from build123d import *

# Parameters (mm, degrees)
EXTRUDE_1_DEPTH              = 13.6
CHAMFER_1_SIZE               = 0.5
HOLE_WIZARD_M4_1_D           = 4.5
HOLE_WIZARD_M4_1_CBORE_D     = 8
HOLE_WIZARD_M4_1_CBORE_DEPTH = 4.4
SKETCH_6_W                   = 2
SKETCH_6_H                   = 15
EXTRUDE_2_DEPTH              = 13.6
HOLE_WIZARD_M3_1_D           = 2.5
MM_1_D                       = 4
MM_1_DEPTH                   = 10
MM_1_TIP                     = 1.201721238
CHAMFER_2_SIZE               = 0.5
MM_2_D                       = 3
MM_2_DEPTH                   = 1
MM_2_TIP                     = 0.901290929


with BuildPart() as part:
    # 草图3 → 凸台-拉伸1 (new body)
    with BuildSketch(Plane.XY):
        Polygon((10, 37.5), (9.5, 38), (-9.5, 38), (-10, 37.5), (-10, 23.5), (-9.5, 23), (-2, 23), (-2, 8), (-9.5, 8), (-10, 7.5), (-10, -7.5), (-9.5, -8), (-2, -8), (-2, -23), (-9.5, -23), (-10, -23.5), (-10, -37.5), (-9.5, -38), (9.5, -38), (10, -37.5), align=None)
    extrude(amount=-EXTRUDE_1_DEPTH)

    # 倒角1
    chamfer_1_edges = [part.edges().sort_by_distance(p)[0] for p in [
        (-10, 30.5, -13.6),
        (-9.75, 37.75, -13.6),
        (0, 38, -13.6),
        (9.75, 37.75, -13.6),
        (10, 0, -13.6),
        (9.75, -37.75, -13.6),
        (-10, -30.5, -13.6),
        (-9.75, -37.75, -13.6),
        (0, -38, -13.6),
        (-10, 30.5, 0),
        (-9.75, 37.75, 0),
        (0, 38, 0),
        (9.75, 37.75, 0),
        (10, 0, 0),
        (9.75, -37.75, 0),
        (-10, -30.5, 0),
        (-9.75, -37.75, 0),
        (0, -38, 0),
    ]]
    chamfer(chamfer_1_edges, length=CHAMFER_1_SIZE)

    # M4 六角凹头螺钉的柱形沉头孔1 (through all)
    with Locations(Plane.ZY.offset(10)):
        with Locations((-6.8, -30), (-6.8, 30)):
            CounterBoreHole(HOLE_WIZARD_M4_1_D / 2, HOLE_WIZARD_M4_1_CBORE_D / 2, HOLE_WIZARD_M4_1_CBORE_DEPTH)

    # 草图6 → 凸台-拉伸2 (add)
    with BuildSketch(Plane.XY):
        with Locations((-3, -15.5)):
            Rectangle(SKETCH_6_W, SKETCH_6_H)
        with Locations((-3, 15.5)):
            Rectangle(SKETCH_6_W, SKETCH_6_H)
    extrude(amount=-EXTRUDE_2_DEPTH)

    # M3 螺纹孔1 (through all)
    with Locations(Plane.ZY.offset(4)):
        with Locations((-6.8, -15.5), (-6.8, 15.5)):
            Hole(HOLE_WIZARD_M3_1_D / 2)

    # 大小mm 暗销孔1
    with Locations(Plane(origin=(10, 0, 0), x_dir=(0, 0, -1), z_dir=(1, 0, 0))):
        with Locations((6.8, -23), (6.8, 23)):
            Hole(MM_1_D / 2, depth=MM_1_DEPTH)
            with Locations((0, 0, -(MM_1_DEPTH + MM_1_TIP / 2))):  # 118° drill point
                Cone(0, MM_1_D / 2, MM_1_TIP, mode=Mode.SUBTRACT)

    # 倒角2
    chamfer_2_edges = [part.edges().sort_by_distance(p)[0] for p in [
        (-10, 30, -10.8),
        (10, 30, -4.55),
        (-10, -30, -10.8),
        (10, -30, -4.55),
        (10, 15.5, -5.55),
        (10, -15.5, -5.55),
        (10, 23, -8.8),
        (10, -23, -8.8),
    ]]
    chamfer(chamfer_2_edges, length=CHAMFER_2_SIZE)

    # 大小mm 暗销孔2
    with Locations(Plane.ZY.offset(10)):
        with Locations((-6.8, 0)):
            Hole(MM_2_D / 2, depth=MM_2_DEPTH)
            with Locations((0, 0, -(MM_2_DEPTH + MM_2_TIP / 2))):  # 118° drill point
                Cone(0, MM_2_D / 2, MM_2_TIP, mode=Mode.SUBTRACT)


solid = part.part
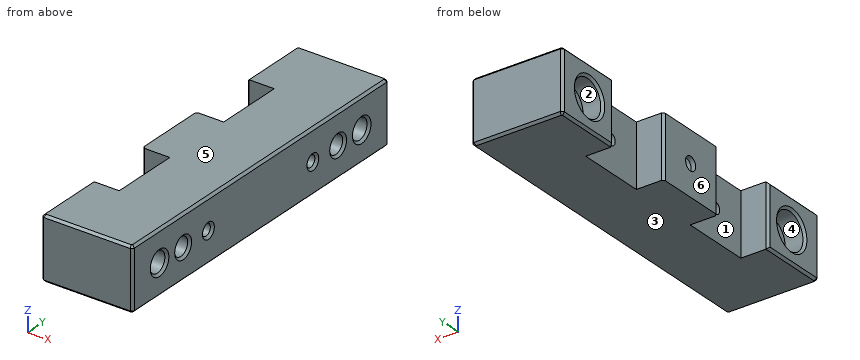
Part model, mm, in its own coordinate system. Face numbers are marked on the shaded views. A direction names the side the tool comes from. Coordinates: 2 decimals unless noted, no trailing zeros. Write each loop counter-clockwise with the first axis right and the second up, starting at its lowest first coordinate (ties: lowest second). Pieces come first, ordered by that corner, then holes. Notation, with made-up numbers: M -17.75,82 L 36.25,82 A23 ccw 36.25,100 Z; hole C 47,66 d1. An arc over 180 degrees is marked long. Return JSON: item names as keys, results as strings.
1. Probe L1, parallel to Y at x = -1.5, z = -6.8; L2, parallel to Y at x = -6.75, z = -6.8; L3, parallel to Z at x = 3.5, y = -23. List the from-to ranges inside material, lowest first.
Determined:
{"L1": "-38 to -32.25, -27.75 to -16.75, -14.25 to 14.25, 16.75 to 27.75, 32.25 to 38", "L2": "-38 to -34, -26 to -23, -8 to 8, 23 to 26, 34 to 38", "L3": "-13.6 to -8.8, -4.8 to 0"}
2. Flat gauge pins, fed straight in: pin 1 Ø3 at (y, z) = (-15.5, -6.8) entering from +X; pin 2 Ø2.5 at (y, z) = (-28, -6) entering from -X; pin 3 Ø4 at (y, z) = (-18.5, -7.5) entering from -X. Where does each tip first touch, or does it go through?
Determined:
{"pin 1": "x = 9.75", "pin 2": "x = -5.6", "pin 3": "x = -4"}
3. Pull direction Z, two halves, no side cores. Call the marked faces 4, 5 and 6: pulls with the +Z half, pulls with the -Z half, needs draft (parallel to the pull), parting line crosses it, or undercut.
Determined:
{"face 4": "undercut", "face 5": "pulls with the +Z half", "face 6": "needs draft"}
4. Saw through at B-B, the plane x = 4. Write the cut outline in (y, z), then the cut area to 3 significant figures.
Determined:
{"outline": "M -38,-13.1 L -37.5,-13.6 L 37.5,-13.6 L 38,-13.1 L 38,-0.5 L 37.5,0 L -37.5,0 L -38,-0.5 Z; hole C -30,-6.8 d4.5; hole C -23,-6.8 d4; hole C -15.5,-6.8 d2.5; hole C 15.5,-6.8 d2.5; hole C 23,-6.8 d4; hole C 30,-6.8 d4.5", "area": "966 mm²"}
5. Saw through at A-A, the plane y = -30. Write the cut outline in (x, z).
Determined:
{"outline": "M -10,-13.1 L -9.5,-13.6 L 9.5,-13.6 L 10,-13.1 L 10,-9.55 L 9.5,-9.05 L -5.6,-9.05 L -5.6,-10.8 L -9.5,-10.8 L -10,-11.3 Z; M -10,-2.3 L -9.5,-2.8 L -5.6,-2.8 L -5.6,-4.55 L 9.5,-4.55 L 10,-4.05 L 10,-0.5 L 9.5,0 L -9.5,0 L -10,-0.5 Z"}
6. Saw through at C-C, the plane y = 15.5. Write the cut outline in (x, z), then the cut area to 3 significant figures.
Determined:
{"outline": "M -4,-13.6 L 9.5,-13.6 L 10,-13.1 L 10,-8.55 L 9.5,-8.05 L -4,-8.05 Z; M -4,-5.55 L 9.5,-5.55 L 10,-5.05 L 10,-0.5 L 9.5,0 L -4,0 Z", "area": "155 mm²"}
7. 3-axis set-ups, long thin cutter, end or side, ignore diameter. For the marked faces 1, 2 and 3: which of +Z, -Z, +X, -X, +Y, -Y reach the whole face in a straight line?
Determined:
{"face 1": "+Z, -Z, -X", "face 2": "-X", "face 3": "-Z, +X, -X, +Y, -Y"}
